The drawing under review shows one solid part. Ordinate dimensions are in mm from its lowest x, y, z. Round coordinates to 2 decimals unless told otherwise and drop trailing zeros. Order: outer loops, then holes, each group sorted by start corner. A loop starts at its lowest first (then second) coordinate and runs counter-clockwise, first axis right, second up. Notation, with made-up numbers: (14, -36) - (31, -36) arc R13 ccw to (31, -28) - close; hole circle Ø6 at (67, 45.5). An arc over 180 degrees is marked (long way). One line per question, with ' | ' between items.
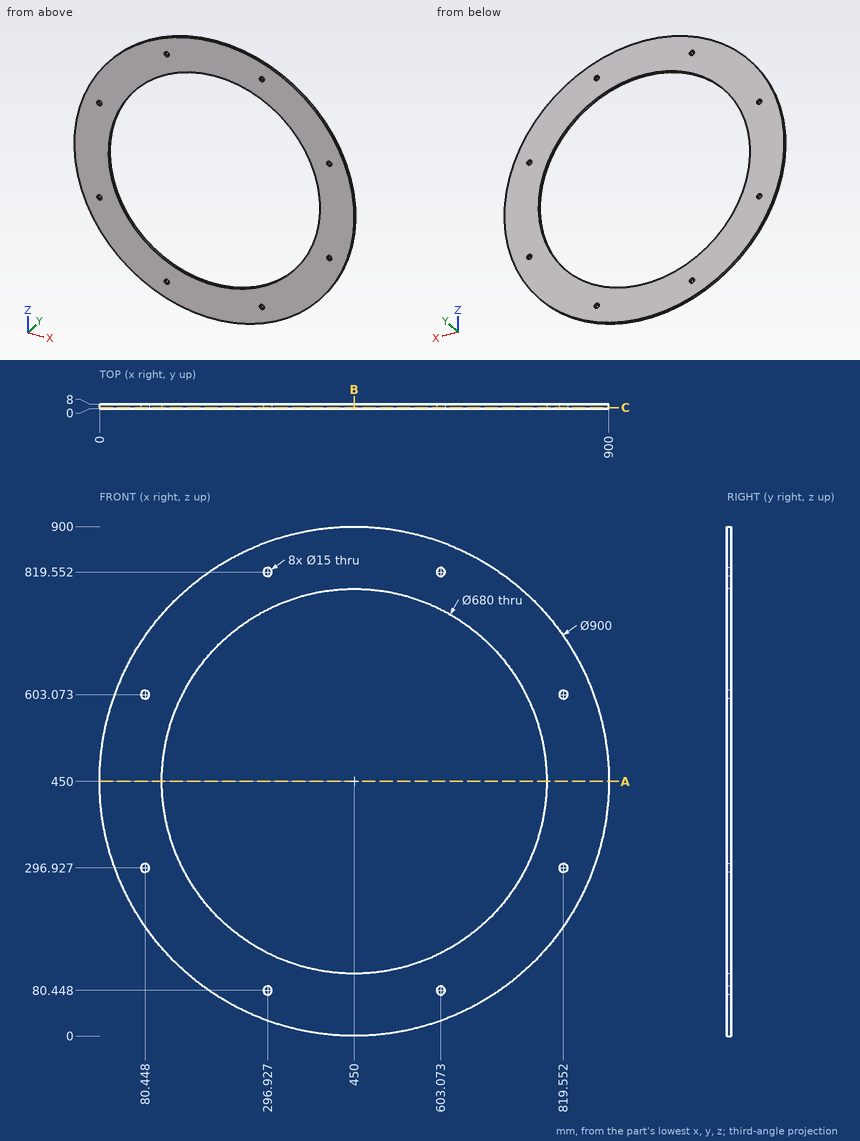
(1) Insertion check: pin 1 (1 mm diameter, centred on y = 4, z = 249.5, fed in from +X); pin 2 (17 mm diameter, centred on x = 80.45, z = 603.07, fed in from -Y); pin 3 (9 mm diameter, centred on x = 603.07, z = 80.45, fed in from +Y). Each pin has a flat end and moves straight along its axis. Give the tip position at first contact, or say it passes through.
Output values:
pin 1: x = 853.11 | pin 2: y = 0 | pin 3: through
(2) We need section B-B on x = 450. State the section outline as (y, z) points, plus the area to 3 significant figures.
Output values:
outline: (0, 0) - (8, 0) - (8, 110) - (0, 110) - close; (0, 790) - (8, 790) - (8, 900) - (0, 900) - close | area: 1,760 mm^2
(3) We need section C-C on y = 1.5. Give the number of separate pieces and of enclosed holes in the cut face, plus the area to 3 significant figures.
Output values:
separate pieces: 1 | enclosed holes: 9 | area: 272,000 mm^2
(4) We need section A-A on z = 450. State the section outline as (x, y) points.
Output values:
outline: (0, 0) - (110, 0) - (110, 8) - (0, 8) - close; (790, 0) - (900, 0) - (900, 8) - (790, 8) - close
(5) For probe 1 along X at (y, z) = (2, 451); probe 2 along Z at (x, y) = (459.5, 7); probe 3 along Z at (x, y) = (196, 2.75), list the stretches that pass through material, from the lowest coordinate up. Write a range as [from, to].
Output values:
probe 1: [0, 110], [790, 900] | probe 2: [0.1, 110.13], [789.87, 899.9] | probe 3: [78.54, 223.98], [676.02, 821.46]
